Design review of the part shown in the three views and the two pictorial views. Dimensions are in mm from the part's minimum x, y and z. Coordinates: 2 decimals unless noted, no trailing zeros. Loops run counter-clockwise (first coordinate to the right, second up) from the corner with the lowest first, then second, coordinate; pieces in that order, holes last. Notation, with made-up numbers: (14.25, 50.25) -> (58.25, 50.25) arc R16 ccw to (58.25, 54.25) -> close; hole circle Ø7 at (87, 47.25). An arc over 180 degrees is marked (long way). Use a Markdown table: item, result. Add a question column.
Q1. Take a section at A-A on x = 211. Write out the cut boundary in (y, z), plus the area to 3 significant figures.
Q2. For probe 1 along X at (y, z) = (110, 12.5) (1 decimal); probe 2 along Y at (x, z) = (225.5, 25.5), list the stretches that pass through material, from the lowest coordinate up.
Q3. Take a section at B-B on z = 23. Write out the cut boundary in (x, y) (1 decimal).
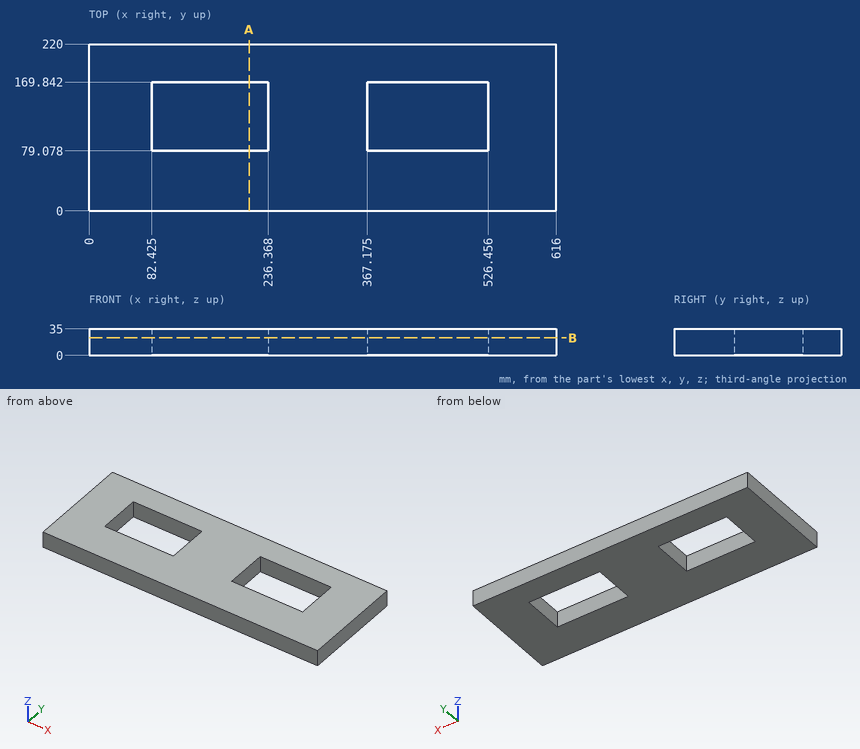
Answer list:
| question | item | result |
|---|---|---|
| 1 | outline | (0, 0) -> (79.08, 0) -> (79.08, 35) -> (0, 35) -> close; (169.84, 0) -> (220, 0) -> (220, 35) -> (169.84, 35) -> close |
| 1 | area | 4,520 mm² |
| 2 | probe 1 | 0 to 82.4, 236.4 to 367.2, 526.5 to 616 |
| 2 | probe 2 | 0 to 79.08, 169.84 to 220 |
| 3 | outline | (0, 0) -> (616, 0) -> (616, 220) -> (0, 220) -> close; hole (82.4, 79.1) -> (236.4, 79.1) -> (236.4, 169.8) -> (82.4, 169.8) -> close; hole (367.2, 79.1) -> (526.5, 79.1) -> (526.5, 169.8) -> (367.2, 169.8) -> close |
